Here's how the part is built. I have some questions about the finished solid (model axes, mm). Face numbers are marked on the shaded views. A direction names the side the tool comes from. Coordinates: 2 decimals unless noted, no trailing zeros. Order: outer loops, then holes, each group sorted by start corner. A loop starts at its lowest first (then second) coordinate and runs counter-clockwise, first axis right, second up. Notation, with made-up numbers: (3, 46.5) - (18, 46.5) arc R24 ccw to (18, 71.5) - close; hole circle Ø11 at (-8.75, 6). An arc over 180 degrees is marked (long way). Answer as CSV lines item,"result". Start each with the question number.
Q1. Suppose I cut it at C-C (x = 144). Please give me the cut outline in (y, z).
Q2. For the marked faces 1 and 2, which set-ups out of +Z, -Z, +X, -X, +Y, -Y let a thin tool reach every point of the face, with its end or its side?
Q3. For pin 1 Ø4 at (y, z) = (-1, -1) entering from -X; pin 2 Ø8 at (x, y) = (120, -6) entering from -Z; pin 3 Ø4 at (x, z) = (152.5, 1) entering from +Y; pin 4 Ø6 at (x, y) = (103, 3) entering from -Z, each with a flat end and sliding along its axis, tell me the tip position at first contact or that it passes through.
Q4. Suppose I cut it at A-A (z = 0). Please give me the cut outline in (x, y).
Q5. I need wall thicknesses on line 1 (X direction, y = 5.75, z = 2.5); line 2 (Y direction, x = 11.5, z = -1.5). Which ranges of each line are inside material? Lowest first, please.
from build123d import *


with BuildPart() as part:
    # Sketch1 → Revolve1 (revolve)
    with BuildSketch(Plane.XY, mode=Mode.PRIVATE) as revolve1_sk:
        Polygon((0, 0), (0, 2.0095), (0.4905, 2.5), (15, 2.5), (15, 2.067), (16.5, 2.067), (16.5, 2.5), (165.5, 2.5), (165.5, 8), (170.5, 8), (170.5, 0), align=None)
    revolve(revolve1_sk.sketch.rotate(Axis((170.5, 0, 0), (-1, 0, 0)), 180), axis=Axis((170.5, 0, 0), (-1, 0, 0)))


solid = part.part
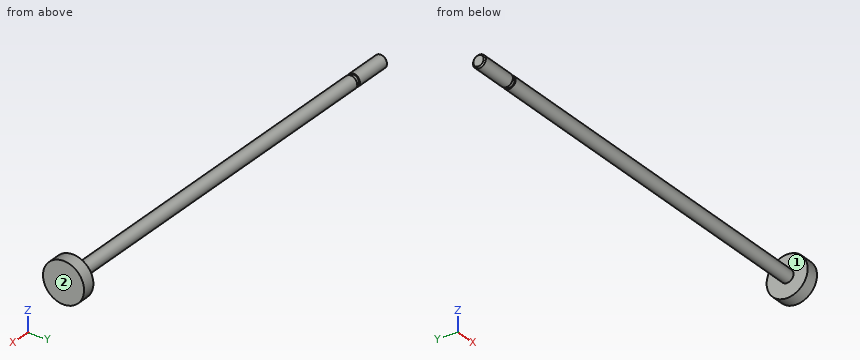
Here are the results:
1,outline,"circle Ø5 at (0, 0)"
2,face 1,"-X"
2,face 2,"+Z, -Z, +X, +Y, -Y"
3,pin 1,"stops at x = 0"
3,pin 2,"stops at z = -1.5"
3,pin 3,"stops at y = 2.5"
3,pin 4,"stops at z = -2.5"
4,outline,"(0, -2.01) - (0.49, -2.5) - (15, -2.5) - (15, -2.07) - (16.5, -2.07) - (16.5, -2.5) - (165.5, -2.5) - (165.5, -8) - (170.5, -8) - (170.5, 8) - (165.5, 8) - (165.5, 2.5) - (16.5, 2.5) - (16.5, 2.07) - (15, 2.07) - (15, 2.5) - (0.49, 2.5) - (0, 2.01) - close"
5,line 1,"x = 165.5 to 170.5"
5,line 2,"y = -2 to 2"
